```python
from build123d import *

# Parameters (mm, degrees)
SKETCH1_W            = 14
SKETCH1_H            = 5
SKETCH3_OUTSIDE_W    = 37.982
SKETCH3_OUTSIDE_H    = 37.982
SKETCH3_OUTSIDE_R    = 9.25
CUT_EXTRUDE2_DEPTH   = 1
M3_CLEARANCE_HOLE1_D = 3.4
SKETCH6_W            = 10
SKETCH6_H            = 31.428384658
CUT_EXTRUDE3_DEPTH   = 1
M4_TAPPED_HOLE1_D    = 3.3
CHAMFER1_SIZE        = 0.5
CHAMFER2_SIZE        = 0.2


with BuildPart() as part:
    # Sketch1 → Revolve1 (revolve)
    with BuildSketch(Plane.XY, mode=Mode.PRIVATE) as revolve1_sk:
        with Locations((7, 2.5)):
            Rectangle(SKETCH1_W, SKETCH1_H)
    revolve(revolve1_sk.sketch.rotate(Axis((0, 0, 0), (0, 1, 0)), 90), axis=Axis((0, 0, 0), (0, 1, 0)))

    # Sketch3 outside → Cut-Extrude2 (cut)
    with BuildSketch(Plane(origin=(0, 5, 0), x_dir=(1, 0, 0), z_dir=(0, 1, 0))):
        Rectangle(SKETCH3_OUTSIDE_W, SKETCH3_OUTSIDE_H)
        with Locations(Location((0, 0, 0), (0, 0, 270))):
            Circle(SKETCH3_OUTSIDE_R, mode=Mode.SUBTRACT)
    extrude(amount=-CUT_EXTRUDE2_DEPTH, mode=Mode.SUBTRACT)

    # M3 Clearance Hole1 (through all)
    with Locations(Plane(origin=(0, 0, 0), x_dir=(-1, 0, 0), z_dir=(0, -1, 0))):
        with Locations((10, -6), (10, 6), (-10, -6), (-10, 6)):
            Hole(M3_CLEARANCE_HOLE1_D / 2)

    # Sketch6 → Cut-Extrude3 (cut)
    with BuildSketch(Plane.XZ):
        Rectangle(SKETCH6_W, SKETCH6_H)
    extrude(amount=-CUT_EXTRUDE3_DEPTH, mode=Mode.SUBTRACT)

    # M4 Tapped Hole1 (through all)
    with Locations(Plane(origin=(0, 1, 0), x_dir=(-1, 0, 0), z_dir=(0, -1, 0))):
        with Locations((0, 0)):
            Hole(M4_TAPPED_HOLE1_D / 2)

    # Chamfer1
    chamfer1_edges = [part.edges().sort_by_distance(p)[0] for p in [
        (0, 4, 14),
        (14, 0, 0),
        (-14, 0, 0),
        (-1.65, 1, 0),
        (-1.65, 5, 0),
    ]]
    chamfer(chamfer1_edges, length=CHAMFER1_SIZE)

    # Chamfer2
    chamfer2_edges = [part.edges().sort_by_distance(p)[0] for p in [
        (0, 5, -9.25),
    ]]
    chamfer(chamfer2_edges, length=CHAMFER2_SIZE)


solid = part.part
```
Model file for the job. Use its own axes, mm. A direction names the side the tool comes from. Coordinates: 2 decimals unless noted, no trailing zeros. Loops run counter-clockwise (first coordinate to the right, second up) from the corner with the lowest first, then second, coordinate; pieces in that order, holes last. Notation, with made-up numbers: (54.5, 78.25) - (86.5, 78.25) arc R21 cw to (86.5, 84.25) - close; hole circle Ø2 at (4, 43.25). An arc over 180 degrees is marked (long way). Answer as a JSON object with one key per item and string values. Group by question number.
(1) Cut at C-C (z = -6). State how many separate pieces and enclosed holes the cut face has, then the cut area to 3 significant figures.
(2) Two-plate mould, pull along X, no slides. Class faces 1 (the face through (-13.64, 0.14, -0.23)), 2 (the face through (9.63, 2.03, -4.34)), 3 (the face through (-2.3, 1, 0.2)), 4 (the face through (9, 4, -3)): released by +X, released by -X, zero draft, split by the parting line, or undercut.
(3) Cut at A-A (z = 0). Give the cut face in (x, y), then the cut area to 3 significant figures.
(4) Probe line 1 along X through (y, z) = (1.95, -6); line 2 along Z through (x, y) = (10, 2.6); line 3 along Z through (x, y) = (-11.25, 2.95). List the from-to ranges inside material, lowest first.
(5) Cut at B-B (x = 0). Give the cut face in (y, z).
(6) Flat gauge pins, fed straight in: pin 1 (0.8 mm diameter, centred on y = 0.5, z = -3.5, fed in from +X); pin 2 (0.8 mm diameter, centred on y = 0.5, z = -2, fed in from -X); pin 3 (5 mm diameter, centred on x = -1.5, z = 1, fed in from -Y). Where does each tip first touch, or does it go through?
(7) Tool access for faces 5 (the face through (9.63, 2.03, 7.66)), 6 (the face through (5, 0.5, -0.2)): list every direction of +Z, -Z, +X, -X, +Y, -Y with a clear straight run to the whole face (end or side of a thin tool).
Geometry says:
{
 "1": {"separate pieces": "3", "enclosed holes": "0", "area": "77.5 mm^2"},
 "2": {"face 1": "released by -X", "face 2": "undercut", "face 3": "undercut", "face 4": "zero draft"},
 "3": {"outline": "(-14, 0.5) - (-13.5, 0) - (-5, 0) - (-5, 1) - (-2.15, 1) - (-1.65, 1.5) - (-1.65, 4.5) - (-2.15, 5) - (-9.05, 5) - (-9.25, 4.8) - (-9.25, 4) - (-13.5, 4) - (-14, 3.5) - close; (1.65, 1.5) - (2.15, 1) - (5, 1) - (5, 0) - (13.5, 0) - (14, 0.5) - (14, 3.5) - (13.5, 4) - (9.25, 4) - (9.25, 4.8) - (9.05, 5) - (2.15, 5) - (1.65, 4.5) - close", "area": "106 mm^2"},
 "4": {"line 1": "x = -12.65 to -11.7, -8.3 to 8.3, 11.7 to 12.65", "line 2": "z = -9.8 to -7.7, -4.3 to 4.3, 7.7 to 9.8", "line 3": "z = -8.33 to -7.15, -4.85 to 4.85, 7.15 to 8.33"},
 "5": {"outline": "(1, -14) - (3.5, -14) - (4, -13.5) - (4, -9.25) - (4.8, -9.25) - (5, -9.05) - (5, -2.15) - (4.5, -1.65) - (1.5, -1.65) - (1, -2.15) - close; (1, 2.15) - (1.5, 1.65) - (4.5, 1.65) - (5, 2.15) - (5, 9.05) - (4.8, 9.25) - (4, 9.25) - (4, 13.5) - (3.5, 14) - (1, 14) - close"},
 "6": {"pin 1": "stops at x = 13.65", "pin 2": "stops at x = -13.91", "pin 3": "stops at y = 1"},
 "7": {"face 5": "+Y, -Y", "face 6": "+Z, -Z, -Y"}
}
